```python
from build123d import *

# Parameters (mm, degrees)
SKETCH_1_W               = 21
SKETCH_1_H               = 6
SKETCH_1_R               = 1.5
EXTRUDE_1_DEPTH          = 6
CUT_EXTRUDE_1_DEPTH      = 23.649503306
CUT_EXTRUDE_1_DEPTH_BACK = 23.649503306
SKETCH_2_R               = 1.5


with BuildPart() as part:
    # 草图1 → 凸台-拉伸1 (new body)
    with BuildSketch(Plane.XY):
        with Locations((10.5, 3)):
            Rectangle(SKETCH_1_W, SKETCH_1_H)
        with Locations((3, 3)):
            Circle(SKETCH_1_R, mode=Mode.SUBTRACT)
        with Locations((13, 3)):
            Circle(SKETCH_1_R, mode=Mode.SUBTRACT)
    extrude(amount=EXTRUDE_1_DEPTH)

    # 草图2 → 切除-拉伸1 (cut, two sides: drawn at the far end of the back side and taken through both)
    with BuildSketch(Plane(origin=(0, 6, 0), x_dir=(1, 0, 0), z_dir=(0, 1, 0)).offset(-CUT_EXTRUDE_1_DEPTH_BACK)):
        with Locations(Location((8, -3, 0), (0, 0, 270))):
            Circle(SKETCH_2_R)
        with Locations(Location((18, -3, 0), (0, 0, 270))):
            Circle(SKETCH_2_R)
    extrude(amount=CUT_EXTRUDE_1_DEPTH + CUT_EXTRUDE_1_DEPTH_BACK, mode=Mode.SUBTRACT)


solid = part.part
```
The listing builds one solid part. Answer for the finished solid, in the listing's coordinates (mm). Round coordinates to 2 decimals unless told otherwise and drop trailing zeros. Write each loop counter-clockwise with the first axis right and the second up, starting at its lowest first coordinate (ties: lowest second). Pieces come first, ordered by that corner, then holes. Notation, with made-up numbers: (48, 2.25) -> (62, 2.25) arc R10 cw to (62, 11.25) -> close; hole circle Ø10 at (18, 18). An arc over 180 degrees is marked (long way). Answer as a JSON object with one key per item and string values. Group by question number.
Q1. Section B-B (z = 3) is taken. Write down the section's boundary in (x, y).
Q2. Section A-A (y = 3) is taken. Write down the section's boundary in (x, z).
Q3. Section C-C (x = 13) is taken. Write down the section's boundary in (y, z), plus the area to 3 significant figures.
Q4. Determine the mould class of faces 1 (the face through (11.8, 2.1, 3)), 2 (the face through (19.265, 2.958, 3.806)), 3 (the face through (10, 6, 3)), 4 (the face through (3.69, 1.67, 2.96)) for opening direction Y: pulls with the +Y half, pulls with the -Y half, needs draft (parallel to the pull), parting line crosses it, or undercut.
Q5. Section D-D (z = 0.55) is taken. Write down the section's boundary in (x, y), plus the area to 3 significant figures.
Q6. Straight lines are drawn through the part: line 1 along X through (y, z) = (1.3, 3); line 2 along X through (y, z) = (2.05, 3); line 3 along X through (y, z) = (3.7, 2.4). For each, find the intervals that lie inside material, in ascending order.
Check values:
{
 "1": {"outline": "(0, 0) -> (6.5, 0) -> (6.5, 6) -> (0, 6) -> close; (9.5, 0) -> (16.5, 0) -> (16.5, 6) -> (9.5, 6) -> close; (19.5, 0) -> (21, 0) -> (21, 6) -> (19.5, 6) -> close; hole circle Ø3 at (3, 3); hole circle Ø3 at (13, 3)"},
 "2": {"outline": "(0, 0) -> (1.5, 0) -> (1.5, 6) -> (0, 6) -> close; (4.5, 0) -> (11.5, 0) -> (11.5, 6) -> (4.5, 6) -> close; (14.5, 0) -> (21, 0) -> (21, 6) -> (14.5, 6) -> close; hole circle Ø3 at (8, 3); hole circle Ø3 at (18, 3)"},
 "3": {"outline": "(0, 0) -> (1.5, 0) -> (1.5, 6) -> (0, 6) -> close; (4.5, 0) -> (6, 0) -> (6, 6) -> (4.5, 6) -> close", "area": "18.0 mm^2"},
 "4": {"face 1": "undercut", "face 2": "needs draft", "face 3": "pulls with the +Y half", "face 4": "undercut"},
 "5": {"outline": "(0, 0) -> (21, 0) -> (21, 6) -> (0, 6) -> close; hole circle Ø3 at (3, 3); hole circle Ø3 at (13, 3)", "area": "112 mm^2"},
 "6": {"line 1": "0 to 6.5, 9.5 to 16.5, 19.5 to 21", "line 2": "0 to 1.84, 4.16 to 6.5, 9.5 to 11.84, 14.16 to 16.5, 19.5 to 21", "line 3": "0 to 1.67, 4.33 to 6.63, 9.37 to 11.67, 14.33 to 16.63, 19.37 to 21"}
}
